Input: dimensioned drawing with shaded views. Units: mm. Origin: part minimum x, y, z. A direction names the side the tool comes from. Round coordinates to 2 decimals unless told otherwise and drop trailing zeros. Order: outer loops, then holes, each group sorted by start corner. A loop starts at its lowest first (then second) coordinate and runs counter-clockwise, first axis right, second up. Notation, with made-up numbers: M 41.25,71.5 L 45.25,71.5 A11 ccw 45.25,81.5 Z; hole C 84,49.25 d9. An arc over 180 degrees is marked long. Answer as CSV lines item,"result". Start each with the question number.
Item 1: First-contact query: P1, Ø10, axis at y = 7.5, z = 67.5, coming from the +X side; P2, Ø3, axis at y = 7.5, z = 30, coming from the -X side. Flat tips, straight axial feed; report the tip coordinate or a pass-through.
Item 2: Line query: line 1 (Y direction, x = 10.25, z = 89.5); line 2 (Y direction, x = 2.5, z = 54.5). Output: solid intervals per line, ascending. Write a range as [from, to].
Item 3: Section query A-A on z = 95.5. Return the cut outline in (x, y).
Item 4: Set-up query: the marked faces 1 and 2. Return all of +Z, -Z, +X, -X, +Y, -Y with unobstructed straight access to the full face (end or side cutting, diameter ignored); none if empty.
Item 5: Section query B-B on y = 26.5. Return the cut outline in (x, z), plus the area to 3 significant figures.
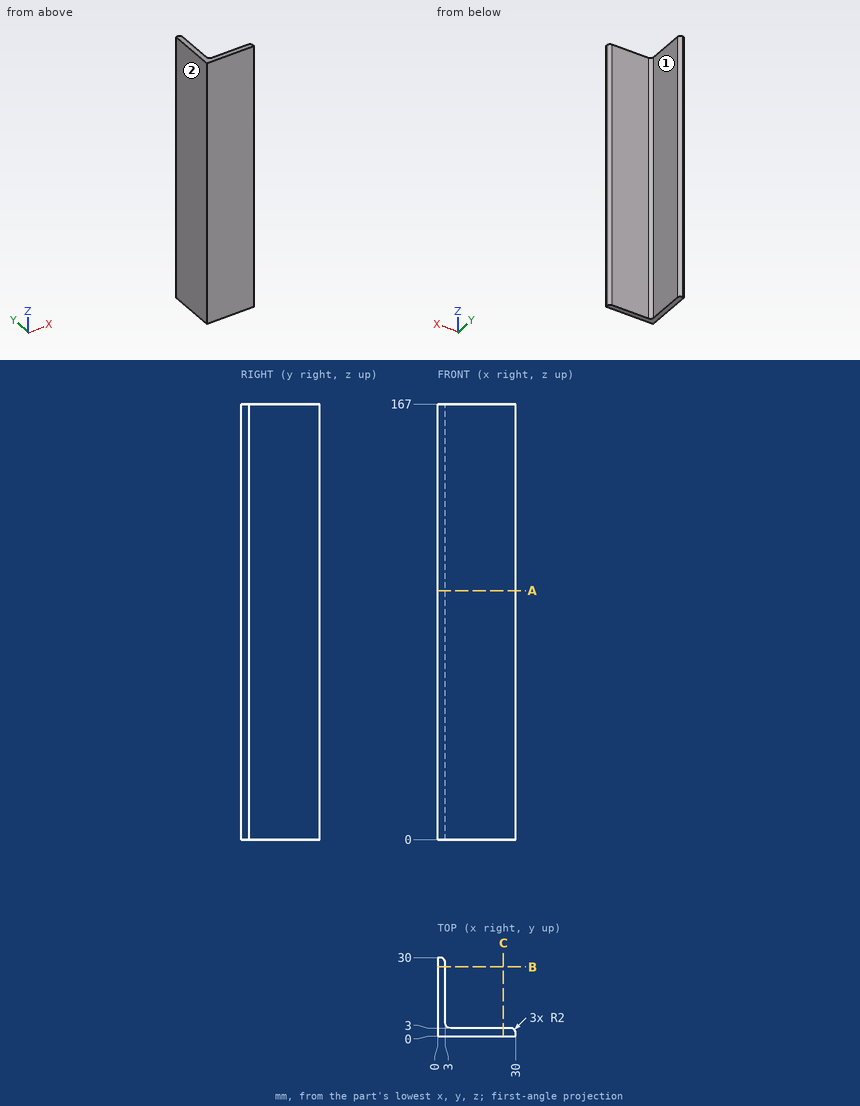
Results:
1,P1,"x = 29.32"
1,P2,"x = 0"
2,line 1,"[0, 3]"
2,line 2,"[0, 29.32]"
3,outline,"M 0,0 L 30,0 L 30,1 A2 ccw 28,3 L 5,3 A2 cw 3,5 L 3,28 A2 ccw 1,30 L 0,30 Z"
4,face 1,"+Z, -Z, +X, +Y"
4,face 2,"+Z, -Z, -X, +Y, -Y"
5,outline,"M 0,0 L 3,0 L 3,167 L 0,167 Z"
5,area,"501 mm^2"
